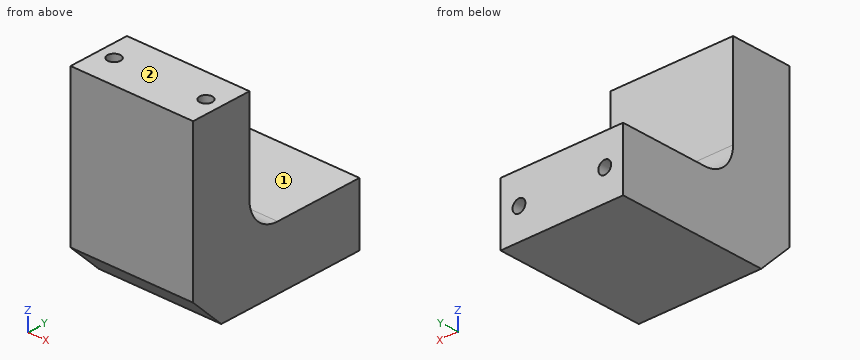
from build123d import *

# Parameters (mm, degrees)
SKETCH1_W             = 40
SKETCH1_H             = 60
BOSS_EXTRUDE1_DEPTH   = 59
SKETCH2_W             = 40
SKETCH2_H             = 39
CUT_EXTRUDE1_DEPTH    = 45
CHAMFER1_SIZE         = 10
FILLET1_R             = 10
M5_TAPPED_HOLE1_D     = 4.2
M5_TAPPED_HOLE1_DEPTH = 12.4
M5_TAPPED_HOLE1_TIP   = 1.2618073
M5_TAPPED_HOLE2_D     = 4.2
M5_TAPPED_HOLE2_DEPTH = 12.4
M5_TAPPED_HOLE2_TIP   = 1.2618073


with BuildPart() as part:
    # Sketch1 → Boss-Extrude1 (new body)
    with BuildSketch(Plane(origin=(0, 0, 0), x_dir=(1, 0, 0), z_dir=(0, 1, 0))):
        Rectangle(SKETCH1_W, SKETCH1_H)
    extrude(amount=BOSS_EXTRUDE1_DEPTH)

    # Sketch2 → Cut-Extrude1 (cut)
    with BuildSketch(Plane(origin=(20, 0, 0), x_dir=(0, 0, -1), z_dir=(1, 0, 0))):
        with Locations((-10, 39.5)):
            Rectangle(SKETCH2_W, SKETCH2_H)
    extrude(amount=-CUT_EXTRUDE1_DEPTH, mode=Mode.SUBTRACT)

    # Chamfer1
    chamfer1_edges = [part.edges().sort_by_distance(p)[0] for p in [
        (0, 0, -30),
    ]]
    chamfer(chamfer1_edges, length=CHAMFER1_SIZE)

    # Fillet1
    fillet1_edges = [part.edges().sort_by_distance(p)[0] for p in [
        (0, 20, -10),
    ]]
    fillet(fillet1_edges, radius=FILLET1_R)

    # M5 Tapped Hole1
    with Locations(Plane(origin=(-14, 59, -20), x_dir=(0, 0, 1), z_dir=(0, 1, 0))):
        with Locations((0, 0), (0, 28)):
            Hole(M5_TAPPED_HOLE1_D / 2, depth=M5_TAPPED_HOLE1_DEPTH)
            with Locations((0, 0, -(M5_TAPPED_HOLE1_DEPTH + M5_TAPPED_HOLE1_TIP / 2))):  # 118° drill point
                Cone(0, M5_TAPPED_HOLE1_D / 2, M5_TAPPED_HOLE1_TIP, mode=Mode.SUBTRACT)

    # M5 Tapped Hole2
    with Locations(Plane(origin=(-15, 10, 30), x_dir=(1, 0, 0), z_dir=(0, 0, 1))):
        with Locations((0, 0), (30, 0)):
            Hole(M5_TAPPED_HOLE2_D / 2, depth=M5_TAPPED_HOLE2_DEPTH)
            with Locations((0, 0, -(M5_TAPPED_HOLE2_DEPTH + M5_TAPPED_HOLE2_TIP / 2))):  # 118° drill point
                Cone(0, M5_TAPPED_HOLE2_D / 2, M5_TAPPED_HOLE2_TIP, mode=Mode.SUBTRACT)


solid = part.part
The listing builds one solid part. Answer for the finished solid, in the listing's coordinates (mm). Face numbers are marked on the shaded views. A direction names the side the tool comes from. Give positions to 0.01 mm unless a question says otherwise; leave off trailing zeros. Write each loop counter-clockwise with the first axis right and the second up, starting at its lowest first coordinate (ties: lowest second). Pieces come first, ordered by that corner, then holes.
1) Given P1, Ø24, axis at x = 8, z = 19.5, coming from the +Y side; P2, Ø1, axis at x = -0.5, y = 29, coming from the +Z side; P3, Ø3.5, axis at x = 15, y = 10, coming from the +Z side; P4, Ø5.5, axis at x = -14, z = -20, coming from the +Y side, each flat-ended and moving along its own axis, determine where each tip first touches the part or whether it passes through.
2) Section B-B (z = 11.5) is taken. Write down the section's boundary in (x, y).
3) Section A-A (x = -5) is taken. Write down the section's boundary in (y, z), and give its area (3 significant figures).
4) Section C-C (y = 39.5) is taken. Write down the section's boundary in (x, z).
5) A tool of negligible diameter and unlimited length cuts with its end or side. For the marked faces 1 and 2, from which of +Z, -Z, +X, -X, +Y, -Y can it reach the whole face along a straight path? Write none if from no direction.
6) Find the intervals of material crossed by L1, parallel to Y at x = 15, z = 20.5; L2, parallel to Z at x = 14, y = 52; L3, parallel to Y at x = -13.5, z = 9.5, in increasing order.
Response:
1. P1: stops at y = 20
1. P2: stops at z = -9.89
1. P3: stops at z = 17.39
1. P4: stops at y = 59
2. outline: (-20, 0) - (20, 0) - (20, 20) - (-20, 20) - close
3. outline: (0, -20) - (10, -30) - (59, -30) - (59, -10) - (30, -10) arc R10 cw to (20, 0) - (20, 30) - (0, 30) - close
3. area: 1,950 mm2
4. outline: (-20, -30) - (20, -30) - (20, -10) - (-20, -10) - close
5. face 1: +Z, +X, -X, +Y
5. face 2: +Z, +X, -X, +Y, -Y
6. L1: y = 0 to 7.9, 12.1 to 20
6. L2: z = -30 to -22.1, -17.9 to -10
6. L3: y = 0 to 20
